from build123d import *

# Parameters (mm, degrees)
END_BORE_30_DEEP_DEPTH = 176.261478164


with BuildPart() as part:
    # Stepped Profile Sketch → Stepped Pulley Body (revolve)
    with BuildSketch(Plane(origin=(0, 0, 0), x_dir=(1, 0, 0), z_dir=(0, 1, 0))):
        Polygon((-80, 15.035517104), (-80, 35.035517104), (-40, 35.035517104), (-40, 42.535517104), (0, 42.535517104), (0, 50.035517104), (40, 50.035517104), (40, 57.535517104), (80, 57.535517104), (80, 49.535517104), (48, 49.535517104), (48, 46.122818691), (8, 46.122818691), (8, 40.273612342), (-32, 40.273612342), (-32, 24.083136151), (40, 24.083136151), (40, 15.035517104), align=None)
    revolve(axis=Axis((40, 0, -15.035517104), (-1, 0, 0)))

    # End Bore Sketch → End Bore 30 Deep (cut, through all)
    with BuildSketch(Plane.ZY.offset(80)):
        with BuildLine():
            Line((-15.035517104, -18), (-12.035517104, -18))
            Line((-12.035517104, -18), (-12.035517104, -14.696938457))
            ThreePointArc((-12.035517104, -14.696938457), (-15.035517104, 15), (-18.035517104, -14.696938457))
            Line((-18.035517104, -14.696938457), (-18.035517104, -18))
            Line((-18.035517104, -18), (-15.035517104, -18))
        make_face()
    extrude(amount=-END_BORE_30_DEEP_DEPTH, mode=Mode.SUBTRACT)


solid = part.part
The model under review builds one solid part; all positions refer to its coordinate system, in mm. A direction names the side the tool comes from. Coordinates: 2 decimals unless noted, no trailing zeros. Write each loop counter-clockwise with the first axis right and the second up, starting at its lowest first coordinate (ties: lowest second). Pieces come first, ordered by that corner, then holes. Notation, with made-up numbers: M 27,49.5 L 77,49.5 A11 cw 77,70.5 Z; hole C 73,21 d1. An arc over 180 degrees is marked long. Put each result on its own line as item: value.
1) Add section D-D on x = 43.5. Give the boundary of the cut face in (y, z).
Computed:
outline: C 0,-15.04 d85; hole C 0,-15.04 d62.17
2) Add section B-B on x = -66. Give the boundary of the cut face in (y, z).
Computed:
outline: C 0,-15.04 d40; hole M -18,-18.04 L -14.7,-18.04 A15 ccw long -14.7,-12.04 L -18,-12.04 Z
3) Draft analysis for pull direction Z (two halves, no side actions). For faces 5 (the flat face through (-32, 11, -26)), 6 (the flat face through (-40, 20.2, -13.1)), 7 (the cylindrical face through (-19.72, 26.846, -9.074)), state which applies: released by +Z, released by -Z, zero draft, split by the parting line, or undercut.
Computed:
face 5: undercut
face 6: zero draft
face 7: split by the parting line
4) Wall thickness on probe 1 along Z at (x, y) = (-45, 0); probe 2 along Y at (x, z) = (29, -14); probe 3 along Z at (x, y) = (-12, 0): over which ranges is each line inside the solid? List them lowest first. Write a range as [from, to].
Computed:
probe 1: z = [-35.04, -30.04], [-0.04, 4.96]
probe 2: y = [-34.98, -31.07], [31.07, 34.98]
probe 3: z = [-42.54, -40.27], [10.2, 12.46]
5) For faces 1 (the cylindrical face through (-12.28, 15.36, 4.99)), 2 (the cylindrical face through (20.28, 31.05, -31.19)), 3 (the flat face through (-56, -16, -12.036)), 4 (the flat face through (-80, 15, -18)), list the 3-axis set-ups (+Z, -Z, +X, -X, +Y, -Y) from which the entire face can be reached by the end or side of a thin tool; tool diameter is ignored.
Computed:
face 1: +X
face 2: -X
face 3: +X, -X
face 4: +Z, -Z, -X, +Y, -Y
6) Clearance check with flat-ended pins moving along their axes: pin 1 Ø3.5 at (x, y) = (-63, -16.5) entering from -Z; pin 2 Ø12 at (x, z) = (52, -47) entering from -Y; pin 3 Ø3.5 at (x, y) = (-54, -16.5) entering from +Z. State where each tip first meets the part, or that it passes through.
Computed:
pin 1: stops at z = -28.54
pin 2: stops at y = -33.65
pin 3: stops at z = -1.53
